from build123d import *

# Parameters (mm, degrees)
SKETCH1_W               = 48
SKETCH1_H               = 16
BOSS_EXTRUDE1_DEPTH     = 20
CUT_EXTRUDE1_DEPTH      = 33.249030993
CUT_EXTRUDE1_DEPTH_BACK = 33.249030993
SKETCH3_R               = 15
BOSS_EXTRUDE2_DEPTH     = 124


with BuildPart() as part:
    # Sketch1 → Boss-Extrude1 (new, symmetric)
    with BuildSketch(Plane(origin=(0, 0, 0), x_dir=(0, 0, -1), z_dir=(1, 0, 0))):
        Rectangle(SKETCH1_W, SKETCH1_H)
    extrude(amount=BOSS_EXTRUDE1_DEPTH, both=True)

    # Sketch2 → Cut-Extrude1 (cut, two sides: drawn at the far end of the back side and taken through both)
    with BuildSketch(Plane(origin=(0, 0, 0), x_dir=(0, 0, -1), z_dir=(1, 0, 0)).offset(-CUT_EXTRUDE1_DEPTH_BACK)):
        Polygon((-24, 8), (-16, -8), (-24, -8), align=None)
        Polygon((24, 8), (24, -8), (16, -8), align=None)
    extrude(amount=CUT_EXTRUDE1_DEPTH + CUT_EXTRUDE1_DEPTH_BACK, mode=Mode.SUBTRACT)

    # Sketch3 → Boss-Extrude2 (add)
    with BuildSketch(Plane.XZ.offset(8)):
        with Locations(Location((0, 0, 0), (0, 0, 90))):
            Circle(SKETCH3_R)
    extrude(amount=BOSS_EXTRUDE2_DEPTH)


solid = part.part
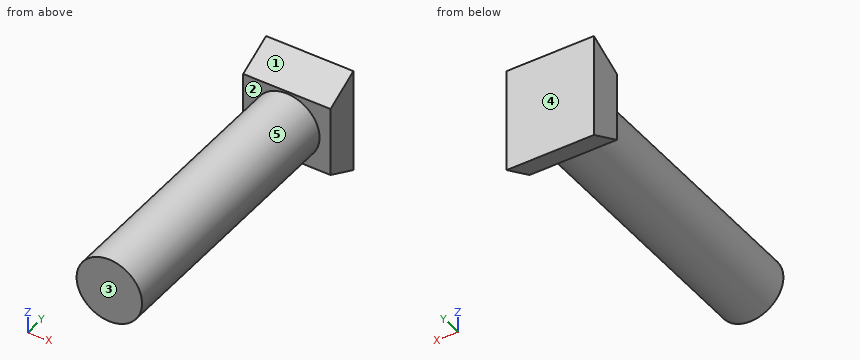
Design review of the part built by this model. Coordinates are the model's own, in mm. Face numbers are marked on the shaded views. A direction names the side the tool comes from. Coordinates: 2 decimals unless noted, no trailing zeros. Order: outer loops, then holes, each group sorted by start corner. A loop starts at its lowest first (then second) coordinate and runs counter-clockwise, first axis right, second up. Notation, with made-up numbers: (66.5, -33.75) -> (72.5, -33.75) arc R29 ccw to (72.5, -11.75) -> close; hole circle Ø4 at (24.25, 35). An arc over 180 degrees is marked (long way). One line per item, written item: value.
1) Clearance check with flat-ended pins moving along their axes: P1, Ø4, axis at y = -15, z = -14.5, coming from the +X side; P2, Ø3, axis at x = -12.5, y = -96.5, coming from the +Z side; P3, Ø10, axis at x = 6.5, y = -37, coming from the +Z side. State where each tip first meets the part, or that it passes through.
Output values:
P1: stops at x = 8.29
P2: stops at z = 10.2
P3: stops at z = 14.92
2) We need section B-B, the plane z = 0. Give the boundary of the cut face in (x, y).
Output values:
outline: (-20, -8) -> (-15, -8) -> (-15, -132) -> (15, -132) -> (15, -8) -> (20, -8) -> (20, 8) -> (-20, 8) -> close
3) Draft analysis for pull direction Y (two halves, no side actions). For the marked faces 3, 4 and 5, state which applies: +Y half, -Y half, draft (parallel to the pull), parting line (faces both ways), or undercut.
Output values:
face 3: -Y half
face 4: +Y half
face 5: draft
4) To check wall thickness, follow probe 1 along Y at (x, z) = (-1, -15); probe 2 along X at (y, z) = (-25, -1); probe 3 along Z at (x, y) = (10.5, -125). State the ranges of each line that lie inside material, in increasing order. Write a range as [from, to].
Output values:
probe 1: y = [-8, 8]
probe 2: x = [-14.97, 14.97]
probe 3: z = [-10.71, 10.71]
5) Machinability: for the marked faces 1 and 2, which of the approach directions +Z, -Z, +X, -X, +Y, -Y give a long, thin tool a straight path to every point of the face, cutting with its end or side? Answer none if there is none.
Output values:
face 1: +Z, +X, -X, -Y
face 2: -Y
6) We need section A-A, the plane x = 0. Give the boundary of the cut face in (y, z).
Output values:
outline: (-132, -15) -> (-8, -15) -> (-8, -16) -> (8, -24) -> (8, 24) -> (-8, 16) -> (-8, 15) -> (-132, 15) -> close
7) We need section C-C, the plane y = -82. Give the boundary of the cut face in (x, z), then the cut area to 3 significant figures.
Output values:
outline: circle Ø30 at (0, 0)
area: 707 mm2
8) We need section D-D, the plane z = -17.5. Give the boundary of the cut face in (x, y).
Output values:
outline: (-20, -5) -> (20, -5) -> (20, 8) -> (-20, 8) -> close
